from build123d import *

# Parameters (mm, degrees)
SKETCH_1_R          = 10
EXTRUDE_1_DEPTH     = 599
CUT_EXTRUDE_START   = 10
CUT_EXTRUDE_3_DEPTH = 3.5


with BuildPart() as part:
    # 草图1 → 凸台-拉伸1 (new, symmetric)
    with BuildSketch(Plane.XY):
        Circle(SKETCH_1_R)
    extrude(amount=EXTRUDE_1_DEPTH, both=True)

    # 草图3 → 切除-拉伸3 (cut)
    with BuildSketch(Plane(origin=(0, 0, 0), x_dir=(1, 0, 0), z_dir=(0, 1, 0)).offset(CUT_EXTRUDE_START)):
        with BuildLine():
            Line((-3, 507), (-3, 545))
            ThreePointArc((-3, 545), (0, 548), (3, 545))
            Line((3, 545), (3, 507))
            ThreePointArc((3, 507), (0, 504), (-3, 507))
        make_face()
        with BuildLine():
            Line((-3, -507), (-3, -545))
            ThreePointArc((-3, -545), (0, -548), (3, -545))
            Line((3, -545), (3, -507))
            ThreePointArc((3, -507), (0, -504), (-3, -507))
        make_face()
        with BuildLine():
            Line((3, 440), (3, 420))
            ThreePointArc((3, 420), (0, 417), (-3, 420))
            Line((-3, 420), (-3, 440))
            ThreePointArc((-3, 440), (0, 443), (3, 440))
        make_face()
        with BuildLine():
            Line((-3, -21), (-3, 17))
            ThreePointArc((-3, 17), (0, 20), (3, 17))
            Line((3, 17), (3, -21))
            ThreePointArc((3, -21), (0, -24), (-3, -21))
        make_face()
    extrude(amount=-CUT_EXTRUDE_3_DEPTH, mode=Mode.SUBTRACT)


solid = part.part
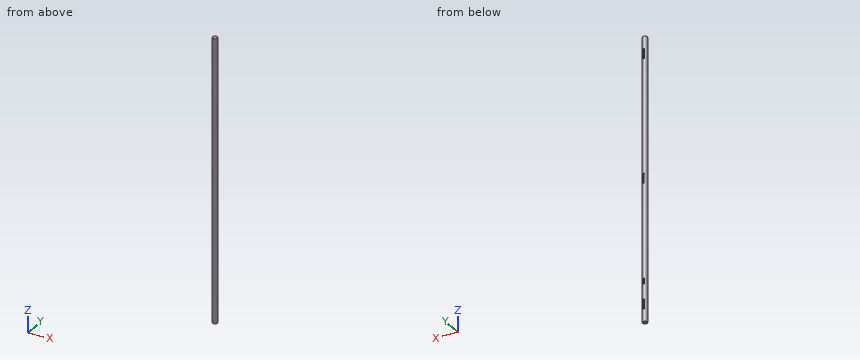
Geometry: final body of the model. Coordinates: model frame, mm. Coordinates: 2 decimals unless noted, no trailing zeros. Loops run counter-clockwise (first coordinate to the right, second up) from the corner with the lowest first, then second, coordinate; pieces in that order, holes last. Notation, with made-up numbers: (-1, -33) - (12, -33) arc R10 cw to (12, -29) - close; hole circle Ø1 at (-25.5, 28.25). An arc over 180 degrees is marked (long way). One line per question, with ' | ' between items. Start each with the question number.
(1) Cut plane B-B on y = -3.5. Output: boundary loops of the cut face in (x, z).
(2) Cut plane A-A on z = 178.5. Output: boundary loops of the cut face in (x, y).
(3) First-contact query: pin 1 (10 mm diameter, centred on x = 7, z = 89, fed in from -Y); pin 2 (2.5 mm diameter, centred on y = 8.5, z = 534.5, fed in from +X); pin 3 (5 mm diameter, centred on x = 1, z = -430, fed in from +Y). Flat tips, straight axial feed; report the tip coordinate or a pass-through.
(4) Ray query, L1, parallel to Z at x = -1, y = 8; L2, parallel to Y at x = -1.5, z = 157.5; L3, parallel to X at y = 2, z = 55. Return the intervals inside material, ascending. Write a range as from..to.
Here are the results:
1) outline: (-9.37, -599) - (9.37, -599) - (9.37, 599) - (-9.37, 599) - close
2) outline: circle Ø20 at (0, 0)
3) pin 1: y = -9.8 | pin 2: x = 6.89 | pin 3: y = 9.54
4) L1: -599..-547.83, -504.17..-442.83, -417.17..-19.83, 23.83..504.17, 547.83..599 | L2: -9.89..9.89 | L3: -9.8..9.8
